Verification items for the finished model (mm, model axes). A direction names the side the tool comes from. Round coordinates to 2 decimals unless told otherwise and drop trailing zeros. Order: outer loops, then holes, each group sorted by start corner. A loop starts at its lowest first (then second) coordinate and runs counter-clockwise, first axis right, second up. Notation, with made-up numbers: (88, 54) -> (107, 54) arc R22 ccw to (107, 81) -> close; hole circle Ø3 at (-2, 23). An arc over 180 degrees is marked (long way). Put each result on its own line as item: value.
```python
from build123d import *

# Parameters (mm, degrees)
SKETCH_2_R                   = 1.6
CUT_EXTRUDE_1_DEPTH          = 30.67322025
CHAMFER_1_SIZE               = 0.5
SKETCH_3_R                   = 3
CUT_EXTRUDE_2_DEPTH          = 3.5
HOLE_WIZARD_M3_1_D           = 2.5
HOLE_WIZARD_M3_1_CSINK_D     = 3.05
HOLE_WIZARD_M3_1_CSINK_ANGLE = 90


with BuildPart() as part:
    # 草图1 → 旋转1 (revolve)
    with BuildSketch(Plane(origin=(0, 0, 0), x_dir=(1, 0, 0), z_dir=(0, 1, 0)), mode=Mode.PRIVATE) as revolve_1_sk:
        Polygon((0, 18.5), (3, 18.5), (3, 17.5), (14, 17.5), (14, 10), (0, 10), align=None)
    revolve(revolve_1_sk.sketch.rotate(Axis((-415.591715209, 0, 0), (1, 0, 0)), 180), axis=Axis((-415.591715209, 0, 0), (1, 0, 0)))

    # 草图2 → 切除-拉伸1 (cut, through all)
    with BuildSketch(Plane(origin=(14, 0, 0), x_dir=(0, 0, -1), z_dir=(1, 0, 0))):
        with Locations((0, 13.5)):
            Circle(SKETCH_2_R)
        with Locations((11.691342951, 6.75)):
            Circle(SKETCH_2_R)
        with Locations((11.691342951, -6.75)):
            Circle(SKETCH_2_R)
        with Locations((0, -13.5)):
            Circle(SKETCH_2_R)
        with Locations((-11.691342951, -6.75)):
            Circle(SKETCH_2_R)
        with Locations((-11.691342951, 6.75)):
            Circle(SKETCH_2_R)
    extrude(amount=-CUT_EXTRUDE_1_DEPTH, mode=Mode.SUBTRACT)

    # 倒角1
    chamfer_1_edges = [part.edges().sort_by_distance(p)[0] for p in [
        (14, 0, -17.5),
    ]]
    chamfer(chamfer_1_edges, length=CHAMFER_1_SIZE)

    # 草图3 → 切除-拉伸2 (cut)
    with BuildSketch(Plane(origin=(14, 0, 0), x_dir=(0, 0, -1), z_dir=(1, 0, 0))):
        with Locations((0, 13.5)):
            Circle(SKETCH_3_R)
        with Locations((11.691342951, 6.75)):
            Circle(SKETCH_3_R)
        with Locations((11.691342951, -6.75)):
            Circle(SKETCH_3_R)
        with Locations((0, -13.5)):
            Circle(SKETCH_3_R)
        with Locations((-11.691342951, -6.75)):
            Circle(SKETCH_3_R)
        with Locations((-11.691342951, 6.75)):
            Circle(SKETCH_3_R)
    extrude(amount=-CUT_EXTRUDE_2_DEPTH, mode=Mode.SUBTRACT)

    # M3 螺纹孔1 (through all)
    with Locations(Plane(origin=(14, 0, 0), x_dir=(0, 0, -1), z_dir=(1, 0, 0))):
        with Locations((-6.75, 11.691342951), (6.75, 11.691342951), (13.5, 0), (6.75, -11.691342951), (-6.75, -11.691342951), (-13.5, 0)):
            CounterSinkHole(HOLE_WIZARD_M3_1_D / 2, HOLE_WIZARD_M3_1_CSINK_D / 2, counter_sink_angle=HOLE_WIZARD_M3_1_CSINK_ANGLE)


solid = part.part
```
Item 1: Tool access check on faces 4 (the face through (12.27, 10.57, 0.65)), 5 (the face through (6.766, -12.452, 5.758)). Record the directions out of +Z, -Z, +X, -X, +Y, -Y that give a thin tool (end or side, any length) a straight path to the whole face; none if there is none.
Geometry check:
face 4: +X
face 5: +X, -X
Item 2: Material ranges on line 1 along Y through (x, z) = (12.45, 0); line 2 along Z through (x, y) = (9.75, 6.5); line 3 along Y through (x, z) = (4.75, -10.5), recorded low to high.
Geometry check:
line 1: -17.5 to -16.5, -10.5 to -10, 10 to 10.5, 16.5 to 17.5
line 2: -16.25 to -13.27, -10.11 to -7.6, 7.6 to 10.11, 13.27 to 16.25
line 3: -14 to -7.82, -5.68 to 5.68, 7.82 to 14
Item 3: Sectioned sample at A-A, the plane y = 0. Record the boundary of the cut face in (x, z) (3 decimals), then the cut area to 3 significant figures.
Geometry check:
outline: (0, -18.5) -> (3, -18.5) -> (3, -17.5) -> (13.5, -17.5) -> (14, -17) -> (14, -15.025) -> (13.725, -14.75) -> (0, -14.75) -> close; (0, -12.25) -> (13.725, -12.25) -> (14, -11.975) -> (14, -10) -> (0, -10) -> close; (0, 10) -> (14, 10) -> (14, 11.975) -> (13.725, 12.25) -> (0, 12.25) -> close; (0, 14.75) -> (13.725, 14.75) -> (14, 15.025) -> (14, 17) -> (13.5, 17.5) -> (3, 17.5) -> (3, 18.5) -> (0, 18.5) -> close
area: 146 mm2
Item 4: Release check for a two-part mould opening along Y. For faces 1 (the face through (10.5, 12, -1)), 2 (the face through (3, 14, -11)), 3 (the face through (8.324, 17.084, -3.794)) record: pulls with the +Y half, pulls with the -Y half, needs draft (parallel to the pull), parting line crosses it, or undercut.
Geometry check:
face 1: undercut
face 2: needs draft
face 3: parting line crosses it
Item 5: Depth check by flat-ended pin: pin 1 Ø12 at (y, z) = (-3.5, 12.5) entering from -X; pin 2 Ø1.5 at (x, y) = (10.5, 14) entering from -Z; pin 3 Ø8 at (x, y) = (3.5, 9.5) entering from -Z; pin 4 Ø5.5 at (y, z) = (-13.5, 0) entering from +X. Enter the tip coordinate at first touch or a pass-through.
Geometry check:
pin 1: x = 0
pin 2: z = -11.43
pin 3: z = -17.65
pin 4: x = 10.5
Item 6: Sectioned sample at B-B, the plane z = 0. Give the number of separate pieces and of enclosed holes in the cut face, then the cut area to 3 significant figures.
Geometry check:
separate pieces: 4
enclosed holes: 0
area: 107 mm2
